Read the model definition and answer for the solid it produces. Units are mm, in the model's axes. A direction names the side the tool comes from. Round coordinates to 2 decimals unless told otherwise and drop trailing zeros. Order: outer loops, then holes, each group sorted by start corner. A loop starts at its lowest first (then second) coordinate and runs counter-clockwise, first axis right, second up. Notation, with made-up numbers: (51, 83) - (73, 83) arc R26 ccw to (73, 100) - close; hole circle Ø2 at (28.25, 40.5). An arc over 180 degrees is marked (long way). One line per question, with ' | ' between items. Start each with the question number.
1) The mould has two halves that part along Y. Classify faces 5 (the cylindrical face through (-77.46, 23.16, -6.69)), 6 (the flat face through (-80, 12, 5)), 7 (the cylindrical face through (-77.46, 23.16, 3.31)), 8 (the flat face through (-1, -35, 0)): pulls with the +Y half, pulls with the -Y half, needs draft (parallel to the pull), parting line crosses it, or undercut.
2) The part is cut by section B-B, the plane x = 0. Give the vertices of the cut face in (y, z).
3) The part is cut by section A-A, the plane y = 20. Give the vertices of the cut face in (x, z), plus the area to 3 significant figures.
4) Straight lines are drawn through the part: line 1 (Y direction, x = 0, z = 1.75); line 2 (Z direction, x = -77, y = 25); line 3 (Y direction, x = -1.5, z = 8.25). For each, find the intervals that lie inside material, in ascending order. Write a range as from..to.
5) The part is cut by section C-C, the plane y = 4. Give the vertices of the cut face in (x, z).
6) For faces 1 (the flat face through (-77, 12, 7)), 2 (the flat face through (-77, 12, 3)), 3 (the flat face through (-77, 12, -6.5)), 4 (the flat face through (-80, 26, -4)), determine the directions among +Z, -Z, +X, -X, +Y, -Y from which every point of the face is accessible in a straight line to the end or side of a thin tool.
7) Flat-ended cylindrical pins translate along their axes: pin 1 (1.5 mm diameter, centred on x = -76.5, y = 12, fed in from +Z); pin 2 (5.5 mm diameter, centred on x = -78.5, y = 12, fed in from -Z); pin 3 (1.5 mm diameter, centred on x = -78.5, z = -4.5, fed in from +Y). Find the tip coordinate at first contact, or state that the pin passes through.
from build123d import *

# Parameters (mm, degrees)
SKETCH2_W           = 150
SKETCH2_H           = 70
BOSS_EXTRUDE1_DEPTH = 10
SKETCH3_R           = 2.5
SKETCH3_R_2         = 1
SKETCH3_W           = 3
SKETCH3_H           = 6
BOSS_EXTRUDE2_DEPTH = 5
CHAMFER1_SIZE       = 2
SKETCH4_R           = 3.5
CUT_EXTRUDE1_DEPTH  = 90.582364336


with BuildPart() as part:
    # Sketch2 → Boss-Extrude1 (new, symmetric)
    with BuildSketch(Plane.XY):
        Rectangle(SKETCH2_W, SKETCH2_H)
    extrude(amount=BOSS_EXTRUDE1_DEPTH, both=True)

    # Sketch3 → Boss-Extrude2 (add)
    # profile 1 of 6: a face of its own
    with BuildSketch(Plane.ZY.offset(75)):
        with Locations(Location((-5, -25, 0), (0, 0, 90))):
            Circle(SKETCH3_R)
        with Locations(Location((-5, -25, 0), (0, 0, 270))):
            Circle(SKETCH3_R_2, mode=Mode.SUBTRACT)
    # profile 2 of 6: a face of its own
    with BuildSketch(Plane.ZY.offset(75)):
        with Locations(Location((5, -25, 0), (0, 0, 90))):
            Circle(SKETCH3_R)
        with Locations(Location((5, -25, 0), (0, 0, 270))):
            Circle(SKETCH3_R_2, mode=Mode.SUBTRACT)
    # profile 3 of 6: a face of its own
    with BuildSketch(Plane.ZY.offset(75)):
        with Locations(Location((5, 25, 0), (0, 0, 90))):
            Circle(SKETCH3_R)
        with Locations(Location((5, 25, 0), (0, 0, 90))):
            Circle(SKETCH3_R_2, mode=Mode.SUBTRACT)
    # profile 4 of 6: a face of its own
    with BuildSketch(Plane.ZY.offset(75)):
        with Locations(Location((-5, 25, 0), (0, 0, 90))):
            Circle(SKETCH3_R)
        with Locations(Location((-5, 25, 0), (0, 0, 90))):
            Circle(SKETCH3_R_2, mode=Mode.SUBTRACT)
    # profile 5 of 6: a face of its own
    with BuildSketch(Plane.ZY.offset(75)):
        with BuildLine():
            Line((7, 13.4135929), (7, 10.4135929))
            ThreePointArc((7, 10.4135929), (5, 8.4135929), (3, 10.4135929))
            Line((3, 10.4135929), (3, 13.4135929))
            ThreePointArc((3, 13.4135929), (5, 15.4135929), (7, 13.4135929))
        make_face()
    # profile 6 of 6: a face of its own
    with BuildSketch(Plane.ZY.offset(75)):
        with Locations((-5, 12)):
            Rectangle(SKETCH3_W, SKETCH3_H)
    extrude(amount=BOSS_EXTRUDE2_DEPTH)

    # Chamfer1
    chamfer1_edges = [part.edges().sort_by_distance(p)[0] for p in [
        (0, -35, 10),
        (75, 0, 10),
        (0, -35, -10),
        (0, 35, -10),
        (75, 0, -10),
        (75, -35, 0),
        (-75, -35, 0),
        (75, 35, 0),
        (0, 35, 10),
    ]]
    chamfer(chamfer1_edges, length=CHAMFER1_SIZE)

    # Sketch4 → Cut-Extrude1 (cut, through all)
    with BuildSketch(Plane.XY.offset(10)):
        with Locations((0, 20)):
            Circle(SKETCH4_R)
        with Locations((0, -20)):
            Circle(SKETCH4_R)
    extrude(amount=-CUT_EXTRUDE1_DEPTH, mode=Mode.SUBTRACT)


solid = part.part
Values:
1) face 5: undercut | face 6: needs draft | face 7: undercut | face 8: pulls with the -Y half
2) outline: (-35, -8) - (-33, -10) - (-23.5, -10) - (-23.5, 10) - (-33, 10) - (-35, 8) - close; (-16.5, -10) - (16.5, -10) - (16.5, 10) - (-16.5, 10) - close; (23.5, -10) - (33, -10) - (35, -8) - (35, 8) - (33, 10) - (23.5, 10) - close
3) outline: (-75, -10) - (-3.5, -10) - (-3.5, 10) - (-75, 10) - close; (3.5, -10) - (73, -10) - (75, -8) - (75, 8) - (73, 10) - (3.5, 10) - close | area: 2,860 mm^2
4) line 1: y = -35..-23.5, -16.5..16.5, 23.5..35 | line 2: z = -7.5..-6, -4..-2.5, 2.5..4, 6..7.5 | line 3: y = -34.75..-23.16, -16.84..16.84, 23.16..34.75
5) outline: (-75, -10) - (73, -10) - (75, -8) - (75, 8) - (73, 10) - (-75, 10) - close
6) face 1: +Z, -X | face 2: -X | face 3: -Z, -X | face 4: +Z, -Z, -X, +Y, -Y
7) pin 1: stops at z = 7 | pin 2: stops at z = -6.5 | pin 3: stops at y = 27.5
